```python
from build123d import *

# Parameters (mm, degrees)
SKETCH_1_W      = 238.5
SKETCH_1_H      = 338.6
SKETCH_1_R      = 1
SKETCH_1_R_2    = 3.55
SKETCH_1_W_2    = 188.5
SKETCH_1_H_2    = 288.6
EXTRUDE_1_DEPTH = 1.5


with BuildPart() as part:
    # 草图1 → 凸台-拉伸1 (new body)
    with BuildSketch(Plane(origin=(2615.929548806, 0, 0), x_dir=(0, 0, -1), z_dir=(1, 0, 0))):
        with Locations((-190.894615796, 1211)):
            Rectangle(SKETCH_1_W, SKETCH_1_H)
        with Locations(Location((-305.144615796, 1046.7, 0), (0, 0, 180))):
            Circle(SKETCH_1_R, mode=Mode.SUBTRACT)
        with Locations(Location((-76.644615796, 1375.3, 0), (0, 0, 180))):
            Circle(SKETCH_1_R, mode=Mode.SUBTRACT)
        with Locations(Location((-289.144615796, 1062.7, 0), (0, 0, 180))):
            Circle(SKETCH_1_R_2, mode=Mode.SUBTRACT)
        with Locations(Location((-92.644615796, 1359.3, 0), (0, 0, 180))):
            Circle(SKETCH_1_R_2, mode=Mode.SUBTRACT)
        with Locations(Location((-92.644615796, 1062.7, 0), (0, 0, 180))):
            Circle(SKETCH_1_R_2, mode=Mode.SUBTRACT)
        with Locations(Location((-289.144615796, 1359.3, 0), (0, 0, 180))):
            Circle(SKETCH_1_R_2, mode=Mode.SUBTRACT)
        with Locations((-190.894615796, 1211)):
            Rectangle(SKETCH_1_W_2, SKETCH_1_H_2, mode=Mode.SUBTRACT)
    extrude(amount=-EXTRUDE_1_DEPTH)


solid = part.part
```
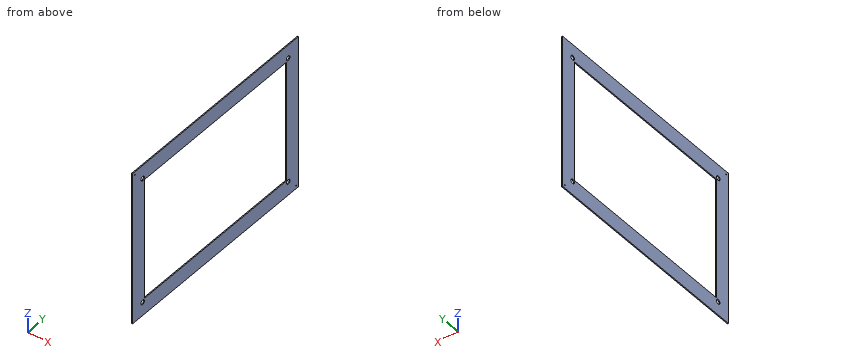
Design review of the part built by this model. Coordinates are the model's own, in mm. Round coordinates to 2 decimals unless told otherwise and drop trailing zeros. Order: outer loops, then holes, each group sorted by start corner. A loop starts at its lowest first (then second) coordinate and runs counter-clockwise, first axis right, second up. Notation, with made-up numbers: (69.25, 19.25) - (114.25, 19.25) arc R18 ccw to (114.25, 42.25) - close; hole circle Ø7 at (1.25, 33). An arc over 180 degrees is marked (long way). Return JSON: item names as keys, results as strings.
Q1. Consider section A-A on y = 1062.7. Write out the cut boundary in (x, z).
Computed values:
{"outline": "(2614.43, 71.64) - (2615.93, 71.64) - (2615.93, 89.09) - (2614.43, 89.09) - close; (2614.43, 96.19) - (2615.93, 96.19) - (2615.93, 285.59) - (2614.43, 285.59) - close; (2614.43, 292.69) - (2615.93, 292.69) - (2615.93, 310.14) - (2614.43, 310.14) - close"}
Q2. Consider section B-B on z = 120. Write out the cut boundary in (x, y), plus the area to 3 significant figures.
Computed values:
{"outline": "(2614.43, 1041.7) - (2615.93, 1041.7) - (2615.93, 1066.7) - (2614.43, 1066.7) - close; (2614.43, 1355.3) - (2615.93, 1355.3) - (2615.93, 1380.3) - (2614.43, 1380.3) - close", "area": "75.0 mm2"}
Q3. For pin 1 Ø5.5 at (y, z) = (1062.7, 289.14) entering from +X, flat-tipped, find the tip position at first contact; note if it passes through.
Computed values:
{"pin 1": "passes through"}
Q4. Wall thickness on L1, parallel to Z at x = 2614.85, y = 1359.3; L2, parallel to Z at x = 2615.35, y = 1315.5; L3, parallel to Y at x = 2614.75, z = 131: over which ranges is each line inside the solid? List them lowest first. Write a range as [from, to].
Computed values:
{"L1": "z = [71.64, 89.09], [96.19, 285.59], [292.69, 310.14]", "L2": "z = [71.64, 96.64], [285.14, 310.14]", "L3": "y = [1041.7, 1066.7], [1355.3, 1380.3]"}
Q5. Consider section D-D on x = 2615.15. Write out the cut boundary in (y, z).
Computed values:
{"outline": "(1041.7, 71.64) - (1380.3, 71.64) - (1380.3, 310.14) - (1041.7, 310.14) - close; hole circle Ø2 at (1046.7, 305.14); hole circle Ø7.1 at (1062.7, 92.64); hole circle Ø7.1 at (1062.7, 289.14); hole (1066.7, 96.64) - (1355.3, 96.64) - (1355.3, 285.14) - (1066.7, 285.14) - close; hole circle Ø7.1 at (1359.3, 92.64); hole circle Ø7.1 at (1359.3, 289.14); hole circle Ø2 at (1375.3, 76.64)"}
Q6. Consider section C-C on y = 1326.5. Write out the cut boundary in (x, z).
Computed values:
{"outline": "(2614.43, 71.64) - (2615.93, 71.64) - (2615.93, 96.64) - (2614.43, 96.64) - close; (2614.43, 285.14) - (2615.93, 285.14) - (2615.93, 310.14) - (2614.43, 310.14) - close"}
